Build history of the part. All positions in model axes, mm. A direction names the side the tool comes from. Round coordinates to 2 decimals unless told otherwise and drop trailing zeros. Write each loop counter-clockwise with the first axis right and the second up, starting at its lowest first coordinate (ties: lowest second). Pieces come first, ordered by that corner, then holes.
1) Flat gauge pins, fed straight in: pin 1 (8 mm diameter, centred on x = 46, z = 2, fed in from -Y); pin 2 (6 mm diameter, centred on x = 144, z = 6, fed in from +Y); pin 3 (5 mm diameter, centred on x = 19, z = 10.5, fed in from -Y). Where does each tip first touch, or does it go through?
2) Saw through at D-D (x = 72.5). Write the cut outline in (y, z).
3) Saw through at B-B (x = 91.5). Write the cut outline in (y, z), plus the area to 3 significant figures.
4) Saw through at C-C (y = 16.5). Write the cut outline in (x, z).
5) Wall check: probe 1 along Y at (x, z) = (97, 1.25); probe 2 along X at (y, z) = (29, 6.5); probe 3 along Y at (x, z) = (74, 9.5). Give the ranges that are in metal, low to high.
6) Which spindle directions (+Z, -Z, +X, -X, +Y, -Y) get a long thin tool onto all of the face, cutting with end or side? Do faces 1 (the flat face through (131.01, -107.14, 7.89)), 2 (the flat face through (180, 147, 6)). Say none if no direction does.
7) Saw through at A-A (z = 3). Write the cut outline in (x, y).
8) Pull direction X, two halves, no side cores. Call faces 3 (the flat face through (51, 2, 0)), 4 (the flat face through (8.89, -113.15, 12.06)), 5 (the flat face through (60, 1, 8)): +X half, -X half, draft (parallel to the pull), parting line (faces both ways), or undercut.
from build123d import *
from OCP.BRepFilletAPI import BRepFilletAPI_MakeChamfer

# Parameters (mm, degrees)
BOSS_EXTRUDE1_DEPTH = 16
CHAMFER1_SIZE       = 10
CHAMFER1_SIZE2      = 12.4055197
CHAMFER2_SIZE       = 8


with BuildPart() as part:
    # Sketch1 → Boss-Extrude1 (new body)
    with BuildSketch(Plane.XY):
        with BuildLine():
            Line((0, -120), (0, 120))
            Line((0, 120), (180, 152.55))
            Line((180, 152.55), (180, 142.864097444))
            ThreePointArc((180, 142.864097444), (176.872536286, 132.125497941), (168.468248072, 124.745356467))
            Line((168.468248072, 124.745356467), (94.595255785, 90.218960551))
            ThreePointArc((94.595255785, 90.218960551), (69.382391143, 68.078536128), (60, 35.862737619))
            Line((60, 35.862737619), (60, -35.762737619))
            ThreePointArc((60, -35.762737619), (69.382391143, -67.978536128), (94.595255785, -90.118960551))
            Line((94.595255785, -90.118960551), (168.468248072, -124.645356467))
            ThreePointArc((168.468248072, -124.645356467), (176.872536286, -132.025497941), (180, -142.764097444))
            Line((180, -142.764097444), (180, -152.55))
            Line((180, -152.55), (0, -120))
        make_face()
    extrude(amount=BOSS_EXTRUDE1_DEPTH)

    # Chamfer1: one chamfer whose edges measure the first distance from different faces: ONE call of the kernel's chamfer builder (chamfer() names one face for all edges)
    chamfer1_edges_1 = [part.edges().sort_by_distance(p)[0] for p in [
        (0, -120, 8),
    ]]
    chamfer1_side_1 = [part.faces().sort_by_distance(p)[0] for p in [
        (0, 0, 8),
    ]]
    chamfer1_edges_2 = [part.edges().sort_by_distance(p)[0] for p in [
        (0, 120, 8),
    ]]
    chamfer1_side_2 = [part.faces().sort_by_distance(p)[0] for p in [
        (90, 136.275, 8),
    ]]
    chamfer1 = BRepFilletAPI_MakeChamfer(part.part.solid().wrapped)
    for e in chamfer1_edges_1:
        chamfer1.Add(CHAMFER1_SIZE, CHAMFER1_SIZE2, e.wrapped, chamfer1_side_1[0].wrapped)  # the first distance lies on this face
    for e in chamfer1_edges_2:
        chamfer1.Add(CHAMFER1_SIZE, CHAMFER1_SIZE2, e.wrapped, chamfer1_side_2[0].wrapped)  # the first distance lies on this face
    add(Compound.cast(chamfer1.Shape()), mode=Mode.REPLACE)

    # Chamfer2
    chamfer2_edges = [part.edges().sort_by_distance(p)[0] for p in [
        (0, -1.20275985, 16),
        (96.103763988, -137.378763988, 16),
        (6.103763988, -116.103763988, 16),
        (4.920200149, 114.686976343, 16),
        (94.920200149, 137.164736194, 16),
    ]]
    chamfer(chamfer2_edges, length=CHAMFER2_SIZE)


solid = part.part
Evaluation:
1. pin 1: stops at y = -129.04
1. pin 2: stops at y = 146.58
1. pin 3: stops at y = -123.48
2. outline: (-133.11, 0) - (-72.42, 0) - (-72.42, 16) - (-124.98, 16) - (-133.11, 8) - close; (72.52, 0) - (133.11, 0) - (133.11, 8) - (124.98, 16) - (72.52, 16) - close
3. outline: (-136.55, 0) - (-88.56, 0) - (-88.56, 16) - (-128.42, 16) - (-136.55, 8) - close; (88.66, 0) - (136.55, 0) - (136.55, 8) - (128.42, 16) - (88.66, 16) - close
3. area: 1,470 mm2
4. outline: (0, 0) - (60, 0) - (60, 16) - (8, 16) - (0, 8) - close
5. probe 1: y = -137.54 to -91.24, 91.34 to 137.54
5. probe 2: x = 0 to 60
5. probe 3: y = -131.86 to -74.29, 74.39 to 131.86
6. face 1: +Z, -Z, +X
6. face 2: +Z, -Z, +X, +Y, -Y
7. outline: (0, -110) - (12.21, -122.21) - (180, -152.55) - (180, -142.76) arc R20 ccw to (168.47, -124.65) - (94.6, -90.12) arc R60 cw to (60, -35.76) - (60, 35.86) arc R60 cw to (94.6, 90.22) - (168.47, 124.75) arc R20 ccw to (180, 142.86) - (180, 152.55) - (9.84, 121.78) - (0, 107.59) - close
8. face 3: draft
8. face 4: -X half
8. face 5: +X half
